Input: part model. Units: mm. Frame: model coordinates. Face numbers are marked on the shaded views. Give positions to 0.01 mm unless a question says otherwise; leave off trailing zeros. Loops run counter-clockwise (first coordinate to the right, second up) from the corner with the lowest first, then second, coordinate; pieces in that order, holes last. Notation, with made-up numbers: M -8,80.25 L 29,80.25 A35 cw 29,112.25 Z; hole C -23,-5.75 d8. An arc over 180 degrees is marked long. Answer as a JSON object with one key per item and string values. Group by question number.
1) Ray query, L1, parallel to Y at x = -49, z = 2.75; L2, parallel to X at y = 86, z = 4.75; L3, parallel to Z at x = 57, y = -108. Return the intervals inside material, ascending.
2) Draft query along Y for the marked faces 1 and 2. Return one class per face: +Y half, -Y half, draft (parallel to the pull), parting line (faces both ways), or undercut.
3) Section query C-C on y = 148.5. Return loops of the section in (x, z).
4) Section query B-B on z = 10. Return loops of the section in (x, y).
5) Section query A-A on y = 21. Return loops of the section in (x, z), plus the area to 3 significant figures.
6) Section query D-D on x = -2.5. Return loops of the section in (y, z).
7) First-contact query: P1, Ø8, axis at x = -138, z = 5, coming from the -Y side; P2, Ø1.1, axis at x = -213.5, z = 19.5, coming from the +Y side; P3, Ø8, axis at x = 147, y = -30.5, coming from the -Z side. Flat tips, straight axial feed; report the tip coordinate or a pass-through.
from build123d import *

# Parameters (mm, degrees)
SKETCH_1_W          = 570
SKETCH_1_H          = 490
EXTRUDE_1_DEPTH     = 20
SHELL_3_T           = -1
SKETCH_5_W          = 570
SKETCH_5_H          = 490
SKETCH_5_W_2        = 550
SKETCH_5_H_2        = 470
EXTRUDE_3_DEPTH     = 1.5
SKETCH_11_R         = 3
EXTRUDE_4_DEPTH     = 10
EXTRUDE_START       = 10
SKETCH_12_R         = 3
EXTRUDE_5_DEPTH     = 10
SKETCH_13_W         = 23
SKETCH_13_H         = 63
CUT_EXTRUDE_3_DEPTH = 1.5


with BuildPart() as part:
    # 草图1 → 凸台-拉伸1 (new body)
    with BuildSketch(Plane.XY):
        Rectangle(SKETCH_1_W, SKETCH_1_H)
    extrude(amount=EXTRUDE_1_DEPTH)

    # 抽壳3
    shell_3_openings = [part.faces().sort_by_distance(p)[0] for p in [
        (0, 0, 0),
    ]]
    offset(amount=SHELL_3_T, openings=shell_3_openings, kind=Kind.INTERSECTION)

    # 草图5 → 凸台-拉伸3 (add)
    with BuildSketch(Plane(origin=(0, 0, 0), x_dir=(-1, 0, 0), z_dir=(0, 0, -1))):
        Rectangle(SKETCH_5_W, SKETCH_5_H)
        Rectangle(SKETCH_5_W_2, SKETCH_5_H_2, mode=Mode.SUBTRACT)
    extrude(amount=-EXTRUDE_3_DEPTH)

    # 草图11 → 凸台-拉伸4 (add)
    with BuildSketch(Plane(origin=(0, 245, 0), x_dir=(1, 0, 0), z_dir=(0, 1, 0))):
        with Locations(Location((275, -10, 0), (0, 0, 90))):
            Circle(SKETCH_11_R)
    extrude(amount=EXTRUDE_4_DEPTH)

    # 草图12 → 凸台-拉伸5 (add)
    with BuildSketch(Plane.XZ.offset(245).offset(EXTRUDE_START)):
        with Locations(Location((275, 10, 0), (0, 0, 270))):
            Circle(SKETCH_12_R)
    extrude(amount=-EXTRUDE_5_DEPTH)

    # 草图13 → 切除-拉伸3 (cut)
    with BuildSketch(Plane.XY.offset(20)):
        with Locations((-213.5, 0)):
            Rectangle(SKETCH_13_W, SKETCH_13_H)
    extrude(amount=-CUT_EXTRUDE_3_DEPTH, mode=Mode.SUBTRACT)


solid = part.part
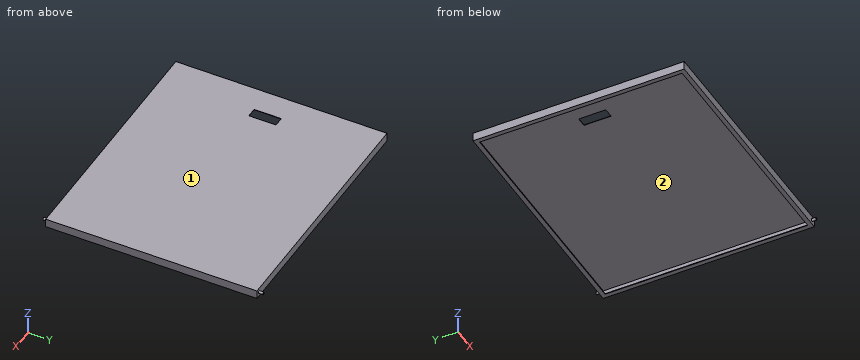
Output:
{
 "1": {"L1": "y = -245 to -244, 244 to 245", "L2": "x = -285 to -284, 284 to 285", "L3": "z = 19 to 20"},
 "2": {"face 1": "draft", "face 2": "undercut"},
 "3": {"outline": "M -285,0 L -275,0 L -275,1.5 L -284,1.5 L -284,19 L 284,19 L 284,1.5 L 275,1.5 L 275,0 L 285,0 L 285,20 L -285,20 Z"},
 "4": {"outline": "M -285,-245 L 272,-245 L 272,-255 L 278,-255 L 278,-245 L 285,-245 L 285,245 L 278,245 L 278,255 L 272,255 L 272,245 L -285,245 Z; hole M -284,-244 L 284,-244 L 284,244 L -284,244 Z"},
 "5": {"outline": "M -285,0 L -275,0 L -275,1.5 L -284,1.5 L -284,19 L -225,19 L -225,20 L -285,20 Z; M -202,19 L 284,19 L 284,1.5 L 275,1.5 L 275,0 L 285,0 L 285,20 L -202,20 Z", "area": "612 mm^2"},
 "6": {"outline": "M -245,0 L -235,0 L -235,1.5 L -244,1.5 L -244,19 L 244,19 L 244,1.5 L 235,1.5 L 235,0 L 245,0 L 245,20 L -245,20 Z"},
 "7": {"P1": "stops at y = -245", "P2": "stops at y = 245", "P3": "stops at z = 19"}
}
